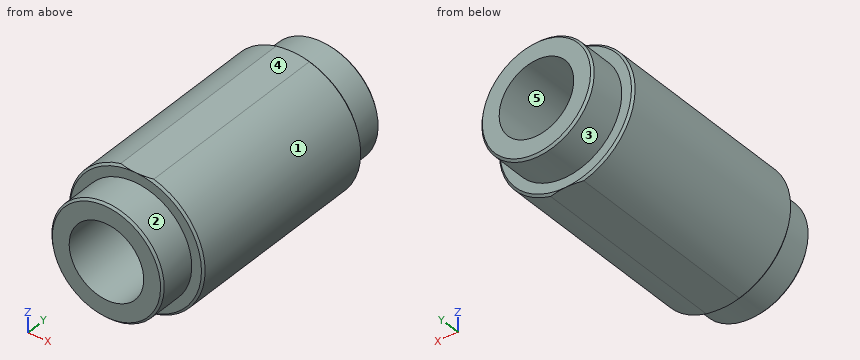
```python
from build123d import *

# Parameters (mm, degrees)
CUT_EXTRUDE1_DEPTH = 251.336773168


with BuildPart() as part:
    # Sketch1 → Revolve1 (revolve)
    with BuildSketch(Plane.XY, mode=Mode.PRIVATE) as revolve1_sk:
        Polygon((-66.5, 230), (-66.5, 38), (-64.5, 36), (-55, 36), (-55, 2), (-53, 0), (-36.5, 0), (-36.5, 268), (-53, 268), (-55, 266), (-55, 232), (-64.5, 232), align=None)
    revolve(revolve1_sk.sketch.rotate(Axis((0, -26.656454657, 0), (0, 1, 0)), 270), axis=Axis((0, -26.656454657, 0), (0, 1, 0)))

    # Sketch2 → Cut-Extrude1 (cut, through all)
    with BuildSketch(Plane.XZ.offset(-36)):
        with BuildLine():
            Line((-16.186414056, 64.5), (16.186414056, 64.5))
            ThreePointArc((16.186414056, 64.5), (0, 66.5), (-16.186414056, 64.5))
        make_face()
        with BuildLine():
            Line((-16.186414056, -64.5), (16.186414056, -64.5))
            ThreePointArc((16.186414056, -64.5), (0, -66.5), (-16.186414056, -64.5))
        make_face()
    extrude(amount=-CUT_EXTRUDE1_DEPTH, mode=Mode.SUBTRACT)


solid = part.part
```
Could you check a few things on this model? Use its own coordinates, in mm. Face numbers are marked on the shaded views. A direction names the side the tool comes from. Round coordinates to 2 decimals unless told otherwise and drop trailing zeros. Loops run counter-clockwise (first coordinate to the right, second up) from the corner with the lowest first, then second, coordinate; pieces in that order, holes last.
Q1. For P1, Ø12, axis at x = -1.5, z = -39, coming from the -Y side; P2, Ø2, axis at x = -34, y = 67.5, coming from the -Z side; P3, Ø10, axis at x = -22.5, y = 157.5, coming from the -Z side; P4, Ø12, axis at y = 152, z = -13, coming from the -X side, each with a flat end and sliding along its axis, tell me the tip position at first contact or that it passes through.
Q2. On a 3-axis mill with a long thin cutter (end or side, diameter ignored), from which of +Z, -Z, +X, -X, +Y, -Y can I reach the whole of each face in a straight line? I mean the marked faces 1 and 2. Say none if no direction works.
Q3. Please list where these lines run through material, in increasing order: L1, parallel to Z at x = 1.5, y = 225; L2, parallel to X at y = 179, z = 0; L3, parallel to Y at x = 24, z = 57.5.
Q4. I want a section at C-C (y = 21.5). Write out the boundary of the cut face in (x, z), and give its area (3 significant figures).
Q5. I want a section at A-A (z = 0). Write out the boundary of the cut face in (x, y).
Q6. I want a section at B-B (y = 177.5). Write out the boundary of the cut face in (x, z), and give its area (3 significant figures).
Q7. Thinking about a two-plate mould opening in X: for the marked faces 3, 4 and 5, which applies, pulls with the +X half, pulls with the -X half, needs draft (parallel to the pull), parting line crosses it, or undercut?
Answer below:
1. P1: stops at y = 0
1. P2: stops at z = -57.73
1. P3: stops at z = -64.16
1. P4: stops at x = -66.13
2. face 1: +X, +Y, -Y
2. face 2: -Y
3. L1: z = -64.5 to -36.47, 36.47 to 64.5
3. L2: x = -66.5 to -36.5, 36.5 to 66.5
3. L3: y = 36 to 232
4. outline: circle Ø110 at (0, 0); hole circle Ø73 at (0, 0)
4. area: 5,320 mm2
5. outline: (-66.5, 38) - (-64.5, 36) - (-55, 36) - (-55, 2) - (-53, 0) - (-36.5, 0) - (-36.5, 268) - (-53, 268) - (-55, 266) - (-55, 232) - (-64.5, 232) - (-66.5, 230) - close; (36.5, 0) - (53, 0) - (55, 2) - (55, 36) - (64.5, 36) - (66.5, 38) - (66.5, 230) - (64.5, 232) - (55, 232) - (55, 266) - (53, 268) - (36.5, 268) - close
6. outline: (-16.19, -64.5) - (16.19, -64.5) arc R66.5 ccw to (16.19, 64.5) - (-16.19, 64.5) arc R66.5 ccw to start; hole circle Ø73 at (0, 0)
6. area: 9,620 mm2
7. face 3: parting line crosses it
7. face 4: needs draft
7. face 5: undercut
